Answer from the drawing. Dimensions are ordinates in mm from the lowest x, y and z of the part. Round coordinates to 2 decimals unless told otherwise and drop trailing zeros. Loops run counter-clockwise (first coordinate to the right, second up) from the corner with the lowest first, then second, coordinate; pieces in that order, holes last. Notation, with made-up numbers: (-0.75, 62.25) - (23.25, 62.25) arc R14 ccw to (23.25, 80.25) - close; hole circle Ø1 at (-40, 80). An arc over 180 degrees is marked (long way). Write item = value, one per line. Start each with the question number.
1) Section C-C, the plane z = 0.15 is taken. Determine the outline of the cut face in (x, y).
2) Given pin 1 Ø3 at (x, y) = (26.5, 5) entering from -Z, flat-ended and moving along its own axis, determine where the tip first touches the part or whether it passes through.
3) Straight lines are drawn through the part: line 1 along X through (y, z) = (12, 0.45); line 2 along X through (y, z) = (6.25, 0.35); line 3 along Z through (x, y) = (12.5, 14.75) (1 decimal). For each, find the intervals that lie inside material, in ascending order.
4) Section A-A, the plane x = 18 is taken. Determine the outline of the cut face in (y, z).
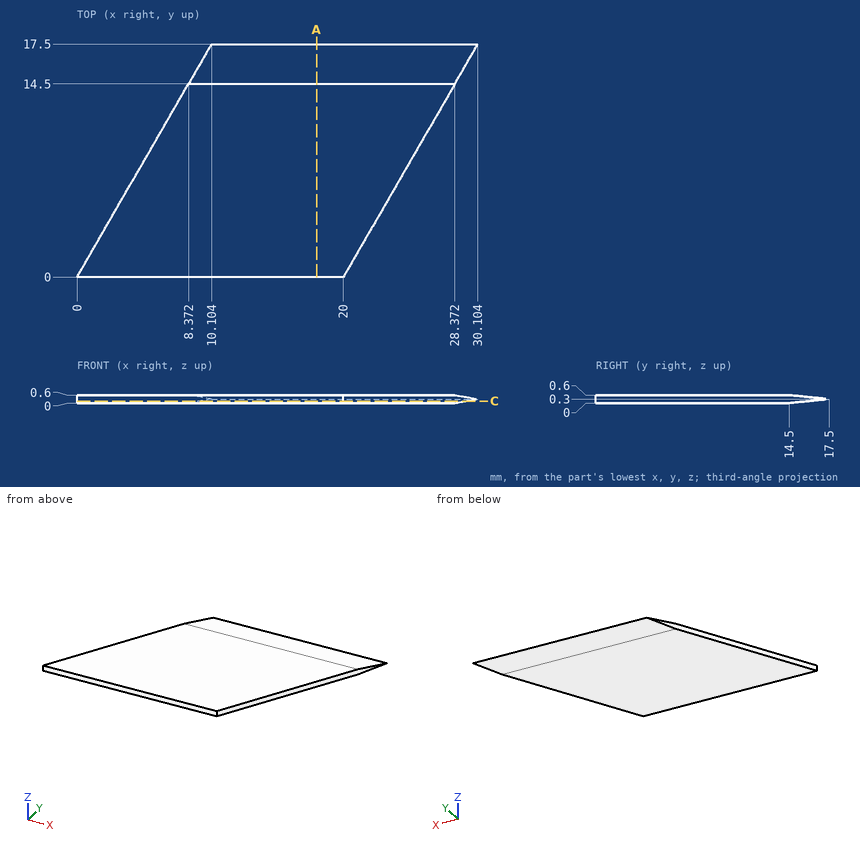
Geometry check:
q1.outline = (0, 0) - (20, 0) - (29.24, 16) - (9.24, 16) - close
q2.pin_1 = through
q3.line_1 = 6.93 to 26.93
q3.line_2 = 3.61 to 23.61
q3.line_3 = 0 to 0.6
q4.outline = (0, 0) - (14.5, 0) - (17.5, 0.3) - (14.5, 0.6) - (0, 0.6) - close
